from build123d import *

# Parameters (mm, degrees)
SKETCH1_R           = 10
SKETCH1_W           = 10
SKETCH1_H           = 10
BOSS_EXTRUDE1_DEPTH = 7.5
SKETCH2_R           = 9
BOSS_EXTRUDE2_DEPTH = 5
CUT_EXTRUDE1_DEPTH  = 38


with BuildPart() as part:
    # Sketch1 → Boss-Extrude1 (new, symmetric)
    with BuildSketch(Plane.XY):
        Circle(SKETCH1_R)
        Rectangle(SKETCH1_W, SKETCH1_H, mode=Mode.SUBTRACT)
    extrude(amount=BOSS_EXTRUDE1_DEPTH, both=True)

    # Sketch2 → Boss-Extrude2 (add, symmetric)
    with BuildSketch(Plane(origin=(0, 0, 0), x_dir=(1, 0, 0), z_dir=(0, 1, 0))):
        with Locations((-35, 16.5)):
            Circle(SKETCH2_R)
        with BuildLine():
            Line((-10, 5.5), (-28.863308582, 23.083389586))
            ThreePointArc((-28.863308582, 23.083389586), (-26.746812047, 20.089552705), (-26, 16.5))
            ThreePointArc((-26, 16.5), (-30.208648574, 8.881407511), (-38.898433669, 8.388143558))
            Line((-38.898433669, 8.388143558), (-10, -5.5))
            Line((-10, -5.5), (-8, -5.5))
            Line((-8, -5.5), (-8, 5.5))
            Line((-8, 5.5), (-10, 5.5))
        make_face()
    boss_extrude2 = extrude(amount=BOSS_EXTRUDE2_DEPTH, both=True)

    # Sketch3 → Cut-Extrude1 (cut, symmetric)
    with BuildSketch(Plane.XY):
        Polygon((-51.292921798, 13.040521839), (-8.660254038, 5), (-44, 2.5), align=None)
        Polygon((-44, -2.5), (-51.292921798, -11.445050359), (-8.660254038, -5), align=None)
    cut_extrude1 = extrude(amount=CUT_EXTRUDE1_DEPTH, both=True, mode=Mode.SUBTRACT)

    # Mirror1: Boss-Extrude2, Cut-Extrude1 across plane
    add(boss_extrude2.mirror(Plane(origin=(0, 0, 0), x_dir=(0, 0, 1), z_dir=(1, 0, 0))))
    add(cut_extrude1.mirror(Plane(origin=(0, 0, 0), x_dir=(0, 0, 1), z_dir=(1, 0, 0))), mode=Mode.SUBTRACT)


solid = part.part
The listing builds one solid part. Answer for the finished solid, in the listing's coordinates (mm). A direction names the side the tool comes from. Round coordinates to 2 decimals unless told otherwise and drop trailing zeros. Order: outer loops, then holes, each group sorted by start corner. A loop starts at its lowest first (then second) coordinate and runs counter-clockwise, first axis right, second up. Notation, with made-up numbers: M 22,46.25 L 72,46.25 A29 cw 72,74.25 Z; hole C -5,24.25 d6. An arc over 180 degrees is marked long. Answer in a Markdown table with one row per item. Add a question column.
1) The part is cut by section B-B on z = -16.5. Determine the outline of the cut face in (x, y).
2) The part is cut by section A-A on x = 0. Determine the outline of the cut face in (y, z).
3) The part is cut by section C-C on z = -1. Determine the outline of the cut face in (x, y), plus the area to 3 significant figures.
4) The part is cut by section D-D on y = -1.5. Determine the outline of the cut face in (x, z).
5) Which of the six approach directions +Z, -Z, +X, -X, +Y, -Y give full straight-line access (tool end or side, diameter ignored) to faces 5 (the face through (-42.31, 0.05, -21.75)), 6 (the face through (5, 0, 0)), 7 (the face through (-19.3, 0.07, -14.17))?
6) Flat-ended cylindrical pins translate along their axes: pin 1 Ø6 at (x, z) = (31.5, -10) entering from +Y; pin 2 Ø5 at (x, y) = (-20.5, 0.5) entering from -Z; pin 3 Ø1.5 at (x, y) = (-9, 3.5) entering from -Z; pin 4 Ø4 at (y, z) = (-6.5, -22) entering from +X. Find the tip coordinate at first contact, or state that the pin passes through.
7) Determine the mould class of faces 1 (the face through (24.65, 0.07, -1.54)), 2 (the face through (-5, 0, 0)), 3 (the face through (-26.083, -3.768, -9.783)), 4 (the face through (0, 5, 0)) for opening direction X: pulls with the +X half, pulls with the -X half, needs draft (parallel to the pull), parting line crosses it, or undercut.
8) Consider line 1 along X through (y, z) = (-2, -13); line 2 along Z through (x, y) = (-1, -6); line 3 along X through (y, z) = (-4, 6). Determine where each line is inside the solid, lowest interval first. Write a range as from..to.
Findings below:
| question | item | result |
|---|---|---|
| 1 | outline | M -44,-2.5 L -21.8,-4.07 L -21.8,4.07 L -44,2.5 Z; M 21.8,-4.07 L 44,-2.5 L 44,2.5 L 21.8,4.07 Z |
| 2 | outline | M -10,-7.5 L -5,-7.5 L -5,7.5 L -10,7.5 Z; M 5,-7.5 L 10,-7.5 L 10,7.5 L 5,7.5 Z |
| 3 | outline | M -23.53,-3.95 L -8.66,-5 A10 ccw 8.66,-5 L 23.53,-3.95 L 23.53,3.95 L 8.66,5 A10 ccw -8.66,5 L -23.53,3.95 Z; hole M -5,-5 L 5,-5 L 5,5 L -5,5 Z |
| 3 | area | 462 mm² |
| 4 | outline | M -38.9,-8.39 A9 ccw long -28.86,-23.08 L -10,-5.5 L -9.89,-5.5 L -9.89,-7.5 L -5,-7.5 L -5,7.5 L -9.89,7.5 L -9.89,5.5 L -10,5.5 Z; M 5,-7.5 L 9.89,-7.5 L 9.89,-5.5 L 10,-5.5 L 28.86,-23.08 A9 ccw long 38.9,-8.39 L 10,5.5 L 9.89,5.5 L 9.89,7.5 L 5,7.5 Z |
| 5 | face 5 | +Y, -Y |
| 5 | face 6 | +Z, -Z |
| 5 | face 7 | -Z, +Y, -Y |
| 6 | pin 1 | stops at y = 3.6 |
| 6 | pin 2 | stops at z = -17.62 |
| 6 | pin 3 | stops at z = -7.5 |
| 6 | pin 4 | passes through |
| 7 | face 1 | pulls with the +X half |
| 7 | face 2 | undercut |
| 7 | face 3 | pulls with the -X half |
| 7 | face 4 | undercut |
| 8 | line 1 | x = -43.29..-18.05, 18.05..43.29 |
| 8 | line 2 | z = -7.5..7.5 |
| 8 | line 3 | x = -9.17..-5, 5..9.17 |
